Job drawing, mm, ordinate dimensions from the low corner. One solid piece. A direction names the side the tool comes from. Round coordinates to 2 decimals unless told otherwise and drop trailing zeros. Order: outer loops, then holes, each group sorted by start corner. A loop starts at its lowest first (then second) coordinate and runs counter-clockwise, first axis right, second up. Notation, with made-up numbers: (62, 42) -> (79, 42) arc R20 ccw to (79, 49) -> close; hole circle Ø9 at (4.5, 34.5). An arc over 180 degrees is marked (long way). Return JSON: item names as keys, results as strings. Group by question number.
Q1. Cut at C-C (y = 1.5). Write the cut outline in (x, z).
Q2. Cut at B-B (x = 10). Write the cut outline in (y, z), then the cut area to 3 significant figures.
Q3. Flat gauge pins, fed straight in: pin 1 (8 mm diameter, centred on y = 6.5, z = 17.5, fed in from -X); pin 2 (3 mm diameter, centred on y = 6, z = 6, fed in from -X); pin 3 (6 mm diameter, centred on x = 17, y = 4.5, fed in from -Z). Where does each tip first touch, or does it go through?
Q4. Which spindle directions (+Z, -Z, +X, -X, +Y, -Y) get a long thin tool onto all of the face, cutting with end or side? Do the marked faces 1 and 2. Say none if no direction does.
Q5. Cut at A-A (z = 10). Write the cut outline in (x, y), then the cut area to 3 significant figures.
Q6. Probe line 1 along Y through (x, z) = (15.25, 14.25); line 2 along Y through (x, z) = (7, 1); line 3 along X through (y, z) = (7.75, 3.5). List the from-to ranges inside material, lowest first.
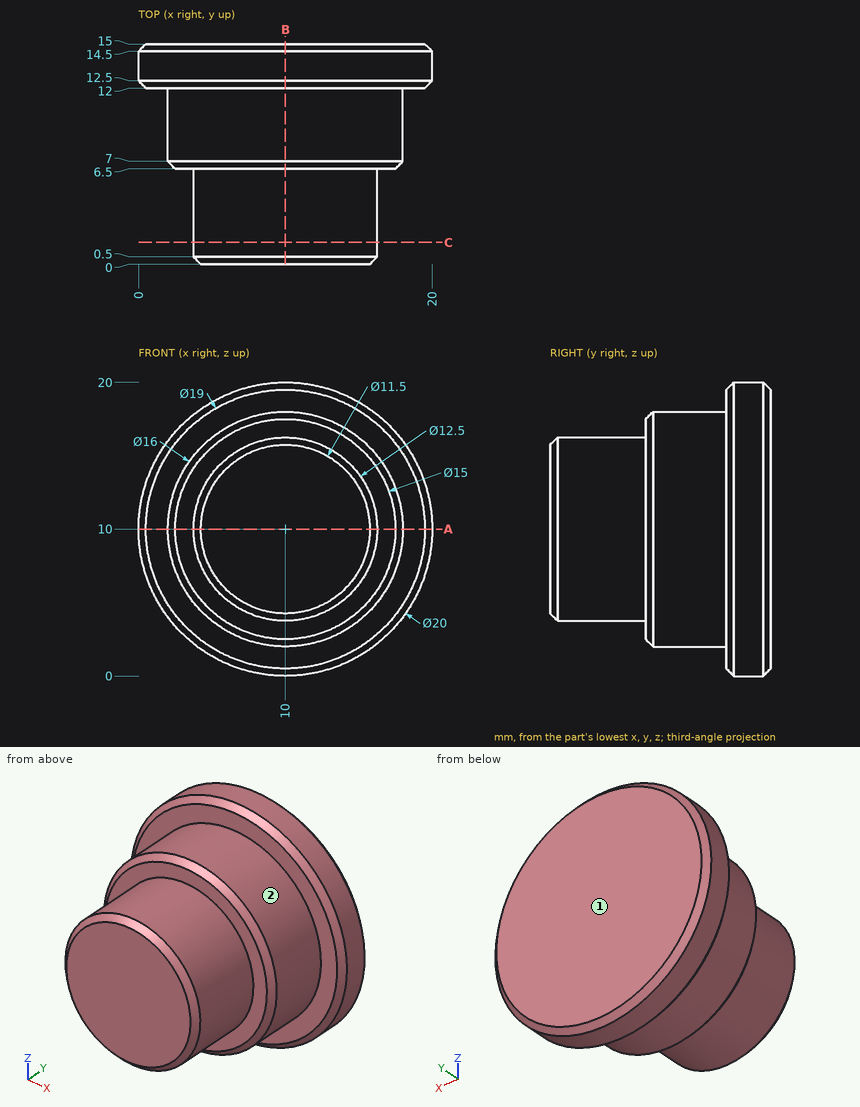
Solution:
{
 "1": {"outline": "circle Ø12.5 at (10, 10)"},
 "2": {"outline": "(0, 4.25) -> (0.5, 3.75) -> (6.5, 3.75) -> (6.5, 2.5) -> (7, 2) -> (12, 2) -> (12, 0.5) -> (12.5, 0) -> (14.5, 0) -> (15, 0.5) -> (15, 19.5) -> (14.5, 20) -> (12.5, 20) -> (12, 19.5) -> (12, 18) -> (7, 18) -> (6.5, 17.5) -> (6.5, 16.25) -> (0.5, 16.25) -> (0, 15.75) -> close", "area": "228 mm²"},
 "3": {"pin 1": "stops at x = 2.82", "pin 2": "stops at x = 2.54", "pin 3": "stops at z = 4.04"},
 "4": {"face 1": "+Z, -Z, +X, -X, +Y", "face 2": "-Y"},
 "5": {"outline": "(0, 12.5) -> (0.5, 12) -> (2, 12) -> (2, 7) -> (2.5, 6.5) -> (3.75, 6.5) -> (3.75, 0.5) -> (4.25, 0) -> (15.75, 0) -> (16.25, 0.5) -> (16.25, 6.5) -> (17.5, 6.5) -> (18, 7) -> (18, 12) -> (19.5, 12) -> (20, 12.5) -> (20, 14.5) -> (19.5, 15) -> (0.5, 15) -> (0, 14.5) -> close", "area": "228 mm²"},
 "6": {"line 1": "y = 6.5 to 15", "line 2": "y = 12 to 15", "line 3": "x = 5.34 to 14.66"}
}
